Can you work these out from the model? Positions are in its coordinate system, mm. Face numbers are marked on the shaded views. A direction names the side the tool comes from. Coordinates: 2 decimals unless noted, no trailing zeros. Write each loop counter-clockwise with the first axis right and the second up, starting at its lowest first coordinate (ties: lowest second). Pieces come first, ordered by that corner, then holes. Notation, with made-up numbers: M 73,-23.5 L 124,-23.5 A30 cw 124,0.5 Z; hole C 29,71 d4. An arc over 180 degrees is marked long. Use one line per item in the form item = value. Start each with the question number.
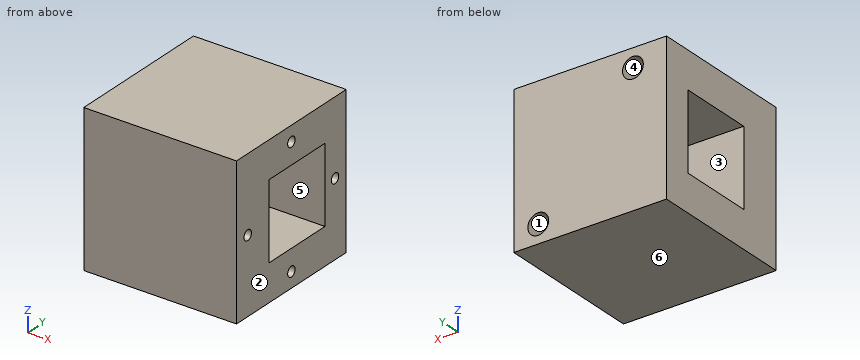
```python
from build123d import *

# Parameters (mm, degrees)
SKETCH_2_W             = 49
SKETCH_2_H             = 49
EXTRUDE_2_DEPTH        = 50
SKETCH_3_W             = 25
SKETCH_3_H             = 25
CUT_EXTRUDE_1_DEPTH    = 50
HOLE_WIZARD_M4_1_D     = 3.3
HOLE_WIZARD_M4_1_DEPTH = 13.5
HOLE_WIZARD_M4_1_TIP   = 0.991420021
HOLE_WIZARD_M8_1_D     = 6.8
HOLE_WIZARD_M8_1_DEPTH = 18
HOLE_WIZARD_M8_1_TIP   = 2.042926105


with BuildPart() as part:
    # 草图2 → 凸台-拉伸2 (new body)
    with BuildSketch(Plane(origin=(0, 0, 0), x_dir=(0, 0, -1), z_dir=(1, 0, 0))):
        with Locations((24.5, 24.5)):
            Rectangle(SKETCH_2_W, SKETCH_2_H)
    extrude(amount=EXTRUDE_2_DEPTH)

    # 草图3 → 切除-拉伸1 (cut)
    with BuildSketch(Plane(origin=(50, 0, 0), x_dir=(0, 0, -1), z_dir=(1, 0, 0))):
        with Locations((24.5, 27)):
            Rectangle(SKETCH_3_W, SKETCH_3_H)
    extrude(amount=-CUT_EXTRUDE_1_DEPTH, mode=Mode.SUBTRACT)

    # M4 螺纹孔1
    with Locations(Plane(origin=(50, 0, 0), x_dir=(0, 0, -1), z_dir=(1, 0, 0))):
        with Locations((24.5, 44), (5, 24.5), (24.5, 5), (44, 24.5)):
            Hole(HOLE_WIZARD_M4_1_D / 2, depth=HOLE_WIZARD_M4_1_DEPTH)
            with Locations((0, 0, -(HOLE_WIZARD_M4_1_DEPTH + HOLE_WIZARD_M4_1_TIP / 2))):  # 118° drill point
                Cone(0, HOLE_WIZARD_M4_1_D / 2, HOLE_WIZARD_M4_1_TIP, mode=Mode.SUBTRACT)

    # M8 螺纹孔1
    with Locations(Plane(origin=(0, 49, 0), x_dir=(-1, 0, 0), z_dir=(0, 1, 0))):
        with Locations((-11, -6), (-42, -43)):
            Hole(HOLE_WIZARD_M8_1_D / 2, depth=HOLE_WIZARD_M8_1_DEPTH)
            with Locations((0, 0, -(HOLE_WIZARD_M8_1_DEPTH + HOLE_WIZARD_M8_1_TIP / 2))):  # 118° drill point
                Cone(0, HOLE_WIZARD_M8_1_D / 2, HOLE_WIZARD_M8_1_TIP, mode=Mode.SUBTRACT)


solid = part.part
```
1) Suppose I cut it at A-A on y = 33. Please give me the cut outline in (x, z), and give its area (3 significant figures).
2) Will these pins go through, and if not, where does the flat tip stop? pin 1 Ø9 at (x, z) = (11, -6) entering from -Y; pin 2 Ø10 at (y, z) = (25, -29) entering from -X.
3) Which directions (+Z, -Z, +X, -X, +Y, -Y) give clear straight access to the entire face, cutting with the end or side of a thin tool? Please do the marked faces 4, 5 and 6.
4) Suppose I cut it at C-C on x = 5.5. Please give me the cut outline in (y, z).
5) If we mould it in two halves opening along X, with no side actions, what happens to the marked faces 1, 2 and 3? For each: +X half, -X half, draft (parallel to the pull), parting line (faces both ways), or undercut.
6) Suppose I cut it at D-D on y = 27.5. Please give me the cut outline in (x, z), and give its area (3 significant figures).
7) Please list where these lines run through material, in increasing order: line 1 (Z direction, x = 11, y = 35.25); line 2 (Y direction, x = 45, z = -24.5); line 3 (Z direction, x = 39, y = 5).
8) Suppose I cut it at B-B on z = -29.5. Please give me the cut outline in (x, y), and give its area (3 significant figures).
Computed values:
q1.outline = M 0,-49 L 50,-49 L 50,-37 L 0,-37 Z; M 0,-12 L 50,-12 L 50,0 L 0,0 Z; hole C 11,-6 d6.8; hole C 42,-43 d6.8
q1.area = 1,130 mm²
q2.pin_1 = 0
q2.pin_2 = through
q3.face_4 = +Y
q3.face_5 = +X, -X
q3.face_6 = -Z, +X, -X, +Y, -Y
q4.outline = M 0,-49 L 49,-49 L 49,0 L 0,0 Z; hole M 14.5,-37 L 39.5,-37 L 39.5,-12 L 14.5,-12 Z
q5.face_1 = undercut
q5.face_2 = +X half
q5.face_3 = draft
q6.outline = M 0,-49 L 50,-49 L 50,-37 L 0,-37 Z; M 0,-12 L 50,-12 L 50,0 L 0,0 Z
q6.area = 1,200 mm²
q7.line_1 = -49 to -37, -12 to -9.4, -2.6 to 0
q7.line_2 = 0 to 3.35, 6.65 to 14.5, 39.5 to 42.35, 45.65 to 49
q7.line_3 = -49 to -26.15, -22.85 to 0
q8.outline = M 0,0 L 50,0 L 50,14.5 L 0,14.5 Z; M 0,39.5 L 50,39.5 L 50,49 L 0,49 Z
q8.area = 1,200 mm²
